```python
from build123d import *

# Parameters (mm, degrees)
SKETCH1_W             = 64
SKETCH1_H             = 25
BOSS_EXTRUDE1_DEPTH   = 40
SKETCH3_R             = 11
SKETCH3_R_2           = 2.5
CUT_EXTRUDE1_DEPTH    = 58
M3_TAPPED_HOLE1_D     = 2.5
M3_TAPPED_HOLE1_DEPTH = 7.5
M3_TAPPED_HOLE1_TIP   = 0.751075774
M8_TAPPED_HOLE1_D     = 6.8
M8_TAPPED_HOLE1_DEPTH = 20
M8_TAPPED_HOLE1_TIP   = 2.042926105
SKETCH11_W            = 15
SKETCH11_H            = 21
SKETCH11_H_2          = 19
CUT_EXTRUDE5_DEPTH    = 58
SKETCH13_R            = 4
SKETCH13_R_2          = 4.1
CUT_EXTRUDE7_DEPTH    = 13
SKETCH14_R            = 4.1
CUT_EXTRUDE8_DEPTH    = 6
SKETCH15_W            = 11.5
SKETCH15_H            = 80
CUT_EXTRUDE11_DEPTH   = 1
SKETCH16_R            = 13.75
CUT_EXTRUDE12_DEPTH   = 4
CHAMFER2_SIZE         = 2
CHAMFER3_SIZE         = 1


with BuildPart() as part:
    # Sketch1 → Boss-Extrude1 (new, symmetric)
    with BuildSketch(Plane.XY):
        Rectangle(SKETCH1_W, SKETCH1_H)
    extrude(amount=BOSS_EXTRUDE1_DEPTH, both=True)

    # Sketch3 → Cut-Extrude1 (cut, through all)
    with BuildSketch(Plane(origin=(0, 12.5, 0), x_dir=(1, 0, 0), z_dir=(0, 1, 0))):
        with Locations(Location((7, 25, 0), (0, 0, 180))):
            Circle(SKETCH3_R)
        with Locations(Location((17, -25, 0), (0, 0, 180))):
            Circle(SKETCH3_R)
        with Locations(Location((-12, 12, 0), (0, 0, 180))):
            Circle(SKETCH3_R_2)
        with Locations(Location((-12, -12, 0), (0, 0, 180))):
            Circle(SKETCH3_R_2)
        with Locations(Location((-26, 12, 0), (0, 0, 180))):
            Circle(SKETCH3_R_2)
        with Locations(Location((-26, -12, 0), (0, 0, 180))):
            Circle(SKETCH3_R_2)
    extrude(amount=-CUT_EXTRUDE1_DEPTH, mode=Mode.SUBTRACT)

    # M3 Tapped Hole1
    with Locations(Plane.ZY.offset(32)):
        with Locations((0, 3.5), (-6, -7.5), (6, -7.5)):
            Hole(M3_TAPPED_HOLE1_D / 2, depth=M3_TAPPED_HOLE1_DEPTH)
            with Locations((0, 0, -(M3_TAPPED_HOLE1_DEPTH + M3_TAPPED_HOLE1_TIP / 2))):  # 118° drill point
                Cone(0, M3_TAPPED_HOLE1_D / 2, M3_TAPPED_HOLE1_TIP, mode=Mode.SUBTRACT)

    # M8 Tapped Hole1
    with Locations(Plane(origin=(0, 12.5, 0), x_dir=(-1, 0, 0), z_dir=(0, 1, 0))):
        with Locations((-12, 0)):
            Hole(M8_TAPPED_HOLE1_D / 2, depth=M8_TAPPED_HOLE1_DEPTH)
            with Locations((0, 0, -(M8_TAPPED_HOLE1_DEPTH + M8_TAPPED_HOLE1_TIP / 2))):  # 118° drill point
                Cone(0, M8_TAPPED_HOLE1_D / 2, M8_TAPPED_HOLE1_TIP, mode=Mode.SUBTRACT)

    # Sketch11 → Cut-Extrude5 (cut, through all)
    with BuildSketch(Plane(origin=(0, 12.5, 0), x_dir=(1, 0, 0), z_dir=(0, 1, 0))):
        with Locations((-24.5, 29.5)):
            Rectangle(SKETCH11_W, SKETCH11_H)
        with Locations((-24.5, -30.5)):
            Rectangle(SKETCH11_W, SKETCH11_H_2)
    extrude(amount=-CUT_EXTRUDE5_DEPTH, mode=Mode.SUBTRACT)

    # Sketch13 → Cut-Extrude7 (cut)
    with BuildSketch(Plane.XZ.offset(12.5)):
        with Locations((-26, -12)):
            Circle(SKETCH13_R)
        with Locations((-26, 12)):
            Circle(SKETCH13_R)
        with Locations((-12, 12)):
            Circle(SKETCH13_R)
        with Locations((-12, -12)):
            Circle(SKETCH13_R)
        with Locations((-26, 0)):
            Circle(SKETCH13_R_2)
    extrude(amount=-CUT_EXTRUDE7_DEPTH, mode=Mode.SUBTRACT)

    # Sketch14 → Cut-Extrude8 (cut)
    with BuildSketch(Plane(origin=(0, 12.5, 0), x_dir=(1, 0, 0), z_dir=(0, 1, 0))):
        with Locations(Location((-12, -12, 0), (0, 0, 180))):
            Circle(SKETCH14_R)
        with Locations(Location((-12, 12, 0), (0, 0, 180))):
            Circle(SKETCH14_R)
    extrude(amount=-CUT_EXTRUDE8_DEPTH, mode=Mode.SUBTRACT)

    # Sketch15 → Cut-Extrude11 (cut)
    with BuildSketch(Plane(origin=(0, -12.5, 0), x_dir=(-1, 0, 0), z_dir=(0, -1, 0))):
        with Locations((11.25, 0)):
            Rectangle(SKETCH15_W, SKETCH15_H)
    extrude(amount=-CUT_EXTRUDE11_DEPTH, mode=Mode.SUBTRACT)

    # Sketch16 → Cut-Extrude12 (cut)
    with BuildSketch(Plane(origin=(0, 12.5, 0), x_dir=(1, 0, 0), z_dir=(0, 1, 0))):
        with Locations(Location((17, -25, 0), (0, 0, 180))):
            Circle(SKETCH16_R)
        with Locations(Location((7, 25, 0), (0, 0, 180))):
            Circle(SKETCH16_R)
    extrude(amount=-CUT_EXTRUDE12_DEPTH, mode=Mode.SUBTRACT)

    # Chamfer2
    chamfer2_edges = [part.edges().sort_by_distance(p)[0] for p in [
        (-17, 0.5, 40),
        (-17, 0.5, -40),
        (32, 0, 40),
        (32, 0, -40),
    ]]
    chamfer(chamfer2_edges, length=CHAMFER2_SIZE)

    # Chamfer3
    chamfer3_edges = [part.edges().sort_by_distance(p)[0] for p in [
        (-32, 0, -19),
        (-32, 0, 21),
    ]]
    chamfer(chamfer3_edges, length=CHAMFER3_SIZE)


solid = part.part
```
Part model, mm, in its own coordinate system. A direction names the side the tool comes from. Coordinates: 2 decimals unless noted, no trailing zeros. Order: outer loops, then holes, each group sorted by start corner. A loop starts at its lowest first (then second) coordinate and runs counter-clockwise, first axis right, second up. Notation, with made-up numbers: (50, -39.5) -> (77, -39.5) arc R17 cw to (77, -15.5) -> close; hole circle Ø11 at (-24.5, 78). An arc over 180 degrees is marked (long way). Put each result on its own line as item: value. Start each with the question number.
(1) Pin check, flat tips, straight feed: pin 1 Ø2 at (y, z) = (-7.5, -6) entering from -X; pin 2 Ø2.5 at (x, z) = (-27.5, 14) entering from -Y; pin 3 Ø5.5 at (x, z) = (12, 0) entering from +Y. Stop position of each tip, or through.
(2) Band-saw the part on D-D (x = -1). Give the cut face in (y, z).
(3) Band-saw the part on C-C (x = 17). Give the cut face in (y, z), then the cut area to 3 significant figures.
(4) Mould opens along Y. For faces 1 (the face through (7.1, 8.5, -13.7)), 2 (the face through (-17, 1, 30)), 3 (the face through (-23.879, 3.715, -0.028)) say: pulls with the +Y half, pulls with the -Y half, needs draft (parallel to the pull), parting line crosses it, or undercut.
(5) Band-saw the part on A-A (z = -25). Give the cut face in (x, y), then the cut area to 4 significant figures.
(6) Band-saw the part on B-B (y = -5). Count the separate pieces of the cut face and the enclosed holes in it, then the cut area to 3 significant figures.
(7) Which spindle directions (+Z, -Z, +X, -X, +Y, -Y) get a long thin tool onto all of the face, cutting with end or side? Do faces 4 (the face through (-11, -11.5, -1)), 5 (the face through (-24, 0.5, -10)), 6 (the face through (0.66, 10.53, -37.2)), 7 (the face through (-24, 0, 21)), 8 (the face through (-28.2, 2.28, 0.27)). Say none if no direction does.
(8) Probe line 1 along Z through (x, y) = (-12, 3.5); line 2 along Z through (x, y) = (-26, 6.75); line 3 along Z through (x, y) = (13, 9). List the from-to ranges inside material, lowest first. Write a range as [from, to].
Determined:
1. pin 1: stops at x = -24.35
1. pin 2: stops at y = 0.5
1. pin 3: stops at y = -7.89
2. outline: (-12.5, -40) -> (12.5, -40) -> (12.5, -36.18) -> (8.5, -36.18) -> (8.5, -32.55) -> (-12.5, -32.55) -> close; (-12.5, -17.45) -> (8.5, -17.45) -> (8.5, -13.82) -> (12.5, -13.82) -> (12.5, 40) -> (-12.5, 40) -> close
3. outline: (-12.5, -40) -> (12.5, -40) -> (12.5, -34.44) -> (8.5, -34.44) -> (8.5, -29.58) -> (-12.5, -29.58) -> close; (-12.5, -20.42) -> (8.5, -20.42) -> (8.5, -15.56) -> (12.5, -15.56) -> (12.5, 11.25) -> (8.5, 11.25) -> (8.5, 14) -> (-12.5, 14) -> close; (-12.5, 36) -> (8.5, 36) -> (8.5, 38.75) -> (12.5, 38.75) -> (12.5, 40) -> (-12.5, 40) -> close
3. area: 1,160 mm²
4. face 1: pulls with the +Y half
4. face 2: needs draft
4. face 3: undercut
5. outline: (-17, -11.5) -> (-5.5, -11.5) -> (-5.5, -12.5) -> (-4, -12.5) -> (-4, 8.5) -> (-6.75, 8.5) -> (-6.75, 12.5) -> (-17, 12.5) -> close; (18, -12.5) -> (32, -12.5) -> (32, 12.5) -> (20.75, 12.5) -> (20.75, 8.5) -> (18, 8.5) -> close
5. area: 641.5 mm²
6. separate pieces: 1
6. enclosed holes: 8
6. area: 3,460 mm²
7. face 4: +Z, -Z, -Y
7. face 5: -Y
7. face 6: +Y
7. face 7: +Z, -X, +Y, -Y
7. face 8: -X
8. line 1: z = [-40, -14.5], [-9.5, 9.5], [14.5, 40]
8. line 2: z = [-19, -14.5], [-9.5, 9.5], [14.5, 21]
8. line 3: z = [-40, -37.37], [-12.63, -3.25], [3.25, 11.84], [38.16, 40]
